The listing builds one solid part. Answer for the finished solid, in the listing's coordinates (mm). Give positions to 0.01 mm unless a question says otherwise; leave off trailing zeros. Order: outer loops, then holes, each group sorted by start corner. A loop starts at its lowest first (then second) coordinate and runs counter-clockwise, first axis right, second up. Notation, with made-up numbers: (-23.5, -6.75) - (-14.5, -6.75) arc R35 ccw to (-14.5, 28.25) - close; hole circle Ø9 at (61, 20). An arc over 180 degrees is marked (long way). Use CSV: the item, a comma, the result in double quotes.
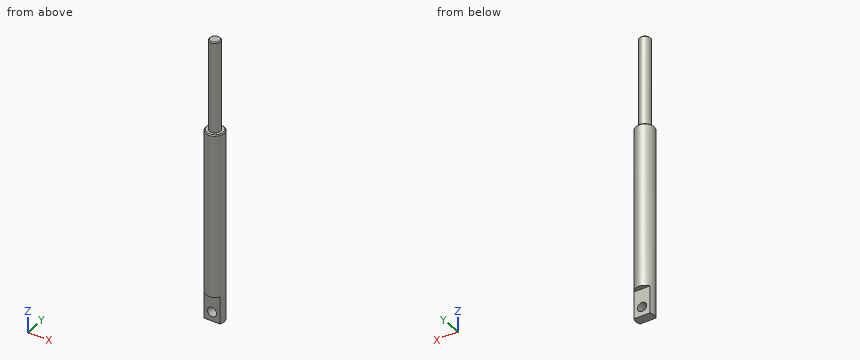
```python
from build123d import *

# Parameters (mm, degrees)
SKETCH1_R               = 10
BOSS_EXTRUDE1_DEPTH     = 210
CUT_EXTRUDE1_DEPTH      = 211.475651798
CUT_EXTRUDE1_DEPTH_BACK = 211.475651798
SKETCH2_R               = 5
CUT_EXTRUDE2_DEPTH      = 211.475651908
CUT_EXTRUDE2_DEPTH_BACK = 30
SKETCH3_W               = 38.012097267
SKETCH3_H               = 10.508452135
SKETCH3_W_2             = 32.719606191
SKETCH3_H_2             = 9.885466079
SKETCH4_R               = 6
BOSS_EXTRUDE2_DEPTH     = 100
CHAMFER1_SIZE           = 1


with BuildPart() as part:
    # Sketch1 → Boss-Extrude1 (new body)
    with BuildSketch(Plane.XY):
        Circle(SKETCH1_R)
    extrude(amount=BOSS_EXTRUDE1_DEPTH)

    # Sketch2 → Cut-Extrude1 (cut, two sides: drawn at the far end of the back side and taken through both)
    with BuildSketch(Plane(origin=(0, 0, 0), x_dir=(1, 0, 0), z_dir=(0, 1, 0)).offset(-CUT_EXTRUDE1_DEPTH_BACK)):
        with Locations(Location((0, -10, 0), (0, 0, 270))):
            Circle(SKETCH2_R)
    extrude(amount=CUT_EXTRUDE1_DEPTH + CUT_EXTRUDE1_DEPTH_BACK, mode=Mode.SUBTRACT)

    # Sketch3 → Cut-Extrude2 (cut, two sides: drawn at the far end of the back side and taken through both)
    with BuildSketch(Plane(origin=(0, 0, 0), x_dir=(-1, 0, 0), z_dir=(0, 0, -1)).offset(-CUT_EXTRUDE2_DEPTH_BACK)):
        with Locations((0.51811282, -10.254226067)):
            Rectangle(SKETCH3_W, SKETCH3_H)
        with Locations((1.092602531, 9.94273304)):
            Rectangle(SKETCH3_W_2, SKETCH3_H_2)
    extrude(amount=CUT_EXTRUDE2_DEPTH + CUT_EXTRUDE2_DEPTH_BACK, mode=Mode.SUBTRACT)

    # Sketch4 → Boss-Extrude2 (add)
    with BuildSketch(Plane.XY.offset(210)):
        Circle(SKETCH4_R)
    extrude(amount=BOSS_EXTRUDE2_DEPTH)

    # Chamfer1
    chamfer1_edges = [part.edges().sort_by_distance(p)[0] for p in [
        (-10, 0, 210),
        (-6, 0, 310),
    ]]
    chamfer(chamfer1_edges, length=CHAMFER1_SIZE)


solid = part.part
```
Item 1: The part is cut by section C-C (z = 10). Give the vertices of the cut face in (x, y), and give its area (3 significant figures).
Taken from the geometry:
outline,"(-8.66, -5) - (-5, -5) - (-5, 5) - (-8.66, 5) arc R10 ccw to start; (5, -5) - (8.66, -5) arc R10 ccw to (8.66, 5) - (5, 5) - close"
area,"91.3 mm^2"
Item 2: The part is cut by section B-B (y = 0). Give the vertices of the cut face in (x, z).
Taken from the geometry:
outline,"(-10, 0) - (10, 0) - (10, 209) - (9, 210) - (6, 210) - (6, 309) - (5, 310) - (-5, 310) - (-6, 309) - (-6, 210) - (-9, 210) - (-10, 209) - close; hole circle Ø10 at (0, 10)"
Item 3: The part is cut by section D-D (z = 251). Give the vertices of the cut face in (x, y), and give its area (3 significant figures).
Taken from the geometry:
outline,"circle Ø12 at (0, 0)"
area,"113 mm^2"
Item 4: Each of these flat-tipped pins is pushed along its axis until it touches: pin 1 (1 mm diameter, centred on x = 6.5, y = -2.5, fed in from +Z); pin 2 (1.5 mm diameter, centred on y = 6, z = 179.5, fed in from -X); pin 3 (5 mm diameter, centred on x = 6.5, z = 235.5, fed in from +Y). Where does it stop, or does it pass through?
Taken from the geometry:
pin 1,"z = 210"
pin 2,"x = -8.51"
pin 3,"y = 4.47"
Item 5: The part is cut by section A-A (x = 0). Give the vertices of the cut face in (y, z), and give its area (3 significant figures).
Taken from the geometry:
outline,"(-10, 30) - (-5, 30) - (-5, 15) - (5, 15) - (5, 30) - (10, 30) - (10, 209) - (9, 210) - (6, 210) - (6, 309) - (5, 310) - (-5, 310) - (-6, 309) - (-6, 210) - (-9, 210) - (-10, 209) - close; (-5, 0) - (5, 0) - (5, 5) - (-5, 5) - close"
area,"5,000 mm^2"
Item 6: Find the intervals of material crossed by line 1 along Z through (x, y) = (0, -2); line 2 along X through (y, z) = (0.75, 10); line 3 along X through (y, z) = (-8, 184.5), in increasing order.
Taken from the geometry:
line 1,"0 to 5, 15 to 310"
line 2,"-9.97 to -5, 5 to 9.97"
line 3,"-6 to 6"
